Verification items for the finished model (mm, model axes). A direction names the side the tool comes from. Coordinates: 2 decimals unless noted, no trailing zeros. Order: outer loops, then holes, each group sorted by start corner. A loop starts at its lowest first (then second) coordinate and runs counter-clockwise, first axis right, second up.
Q1. Cross-section at C-C, the plane x = 29. Record the boundary of the cut face in (y, z).
Q2. Set-up check for faces 1 (the flat face through (35, 79, -91)), 2 (the flat face through (5, 142, 3)), 3 (the cylindrical face through (25.14, 82.15, -107.13)): record each of +Z, -Z, +X, -X, +Y, -Y from which the full face is reachable in a straight line by a thin tool's end or side.
Q3. Thickness scan on line 1 (Y direction, x = 13, z = 0); line 2 (Y direction, x = 25, z = 0); line 3 (X direction, y = 154, z = 95.5). Record the ranges inside material, lowest first.
Q4. Cross-section at D-D, the plane y = -190.5. Record the boundary of the cut face in (x, z), and give its area (3 significant figures).
Q5. Draft check along X on faces 4 (the conical face through (3.75, 117.39, -26.07)), 5 (the cylindrical face through (10.07, -65.481, 207.933)), 6 (the flat face through (15, 94, -100)). Enter one of: pulls with the +X half, pulls with the -X half, needs draft (parallel to the pull), parting line crosses it, or undercut.
Q6. Depth check by flat-ended pin: P1, Ø10, axis at x = 26, z = -58.5, coming from the +Y side; P2, Ø5, axis at x = 11, z = 154, coming from the +Y side; P3, Ø6, axis at x = 22.5, y = -123, coming from the +Z side. Enter the tip coordinate at first touch or a pass-through.
Q7. Cross-section at A-A, the plane y = 0. Record the boundary of the cut face in (x, z), and give its area (3 significant figures).
from build123d import *

# Parameters (mm, degrees)
CHAMFER1_SIZE = 4


with BuildPart() as part:
    # Sketch1 → Revolve1 (revolve)
    with BuildSketch(Plane.XY, mode=Mode.PRIVATE) as revolve1_sk:
        Polygon((0, 140), (5, 140), (5, 218), (15, 218), (15, 135), (35, 135), (35, 120), (0, 120), align=None)
    revolve(revolve1_sk.sketch.rotate(Axis((0, 0, 0), (1, 0, 0)), 90), axis=Axis((0, 0, 0), (1, 0, 0)))

    # Chamfer1
    chamfer1_edges = [part.edges().sort_by_distance(p)[0] for p in [
        (0, 0, -120),
    ]]
    chamfer(chamfer1_edges, length=CHAMFER1_SIZE)


solid = part.part
Check values:
1. outline: circle Ø270 at (0, 0); hole circle Ø240 at (0, 0)
2. face 1: +Z, -Z, +X, +Y, -Y
2. face 2: -X
2. face 3: +X
3. line 1: y = -218 to -120, 120 to 218
3. line 2: y = -135 to -120, 120 to 135
3. line 3: x = 5 to 15
4. outline: (5, -105.99) - (15, -105.99) - (15, 105.99) - (5, 105.99) - close
4. area: 2,120 mm2
5. face 4: pulls with the -X half
5. face 5: needs draft
5. face 6: pulls with the +X half
6. P1: stops at y = 123.95
6. P2: stops at y = 156.75
6. P3: stops at z = 61.85
7. outline: (0, -140) - (5, -140) - (5, -218) - (15, -218) - (15, -135) - (35, -135) - (35, -120) - (4, -120) - (0, -124) - close; (0, 124) - (4, 120) - (35, 120) - (35, 135) - (15, 135) - (15, 218) - (5, 218) - (5, 140) - (0, 140) - close
7. area: 2,740 mm2
